The figure shows three views and two pictorial views of one solid part (mm, origin at its lowest corner). Answer the questions. Give positions to 0.01 mm unless a question says otherwise; leave off trailing zeros. Write each loop counter-clockwise with the first axis right and the second up, starting at its lowest first coordinate (ties: lowest second). Pieces come first, ordered by that corner, then holes. Notation, with made-up numbers: (22.5, 69.25) -> (75.5, 69.25) arc R16 cw to (75.5, 94.25) -> close; hole circle Ø4 at (-39.5, 19). An arc over 180 degrees is marked (long way). Answer as CSV lines item,"result". Start each with the question number.
1. The part is cut by section D-D, the plane y = 31. Determine the outline of the cut face in (x, z), and give its area (3 significant figures).
2. The part is cut by section B-B, the plane z = 47.5. Determine the outline of the cut face in (x, y).
3. The part is cut by section A-A, the plane x = 47.5. Determine the outline of the cut face in (y, z), and give its area (3 significant figures).
4. The part is cut by section C-C, the plane y = 9.5. Determine the outline of the cut face in (x, z).
5. For a pull along Z with two mould halves and no side action, classify the marked faces 1, 2, 3 and 4 as pulls with the +Z half, pulls with the -Z half, needs draft (parallel to the pull), parting line crosses it, or undercut.
6. Find the intervals of material crossed by line 1 (X direction, y = 28, z = 47); line 2 (X direction, y = 26, z = 47); line 3 (Y direction, x = 89, z = 58), in increasing order.
7. Given pin 1 (1 mm diameter, centred on x = 24, z = 78.5, fed in from -Y); pin 2 (2 mm diameter, centred on x = 29.5, y = 4.5, fed in from -Z); pin 3 (1.5 mm diameter, centred on y = 13.5, z = 69.5, fed in from +X), each flat-ended and moving along its own axis, determine where each tip first touches the part or whether it passes through.
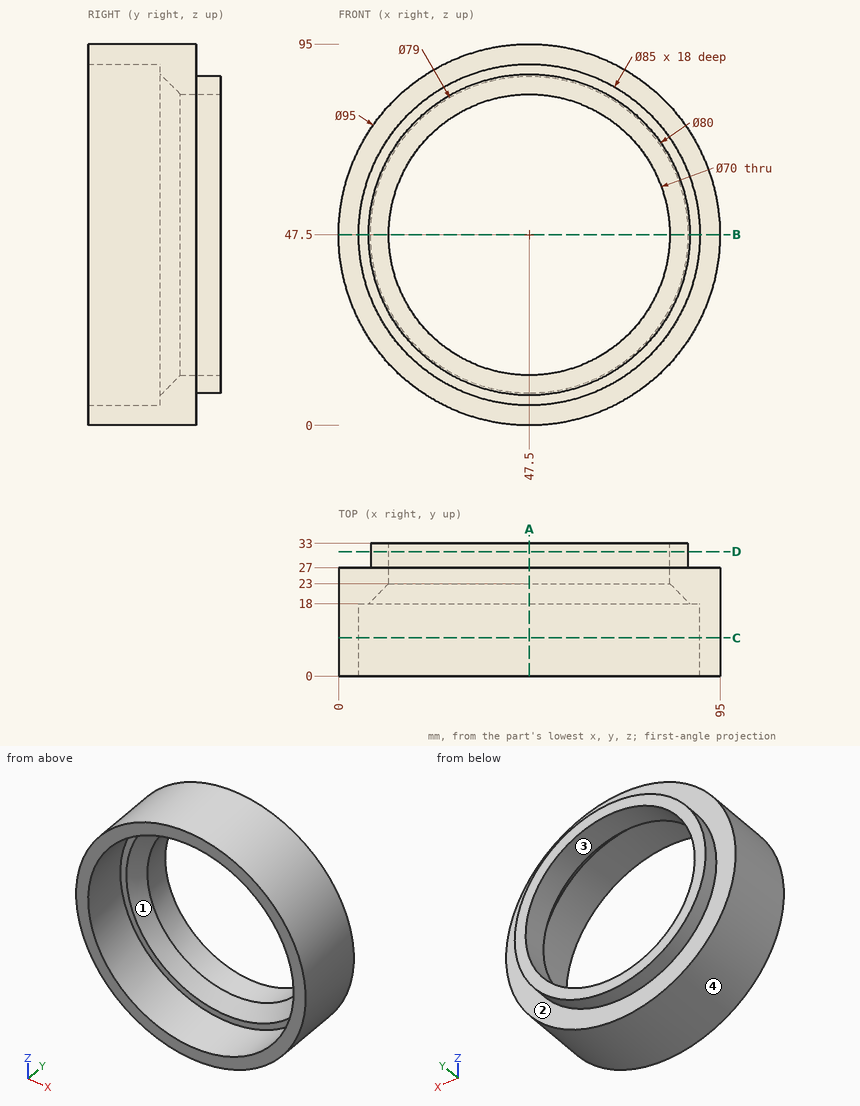
Results found:
1,outline,"circle Ø79 at (47.5, 47.5); hole circle Ø70 at (47.5, 47.5)"
1,area,"1,050 mm²"
2,outline,"(0, 0) -> (5, 0) -> (5, 18) -> (7.5, 18) -> (12.5, 23) -> (12.5, 33) -> (8, 33) -> (8, 27) -> (0, 27) -> close; (82.5, 23) -> (87.5, 18) -> (90, 18) -> (90, 0) -> (95, 0) -> (95, 27) -> (87, 27) -> (87, 33) -> (82.5, 33) -> close"
3,outline,"(0, 0) -> (27, 0) -> (27, 8) -> (33, 8) -> (33, 12.5) -> (23, 12.5) -> (18, 7.5) -> (18, 5) -> (0, 5) -> close; (0, 90) -> (18, 90) -> (18, 87.5) -> (23, 82.5) -> (33, 82.5) -> (33, 87) -> (27, 87) -> (27, 95) -> (0, 95) -> close"
3,area,"434 mm²"
4,outline,"circle Ø95 at (47.5, 47.5); hole circle Ø85 at (47.5, 47.5)"
5,face 1,"undercut"
5,face 2,"needs draft"
5,face 3,"undercut"
5,face 4,"parting line crosses it"
6,line 1,"x = 8 to 12.5, 82.5 to 87"
6,line 2,"x = 0 to 12.5, 82.5 to 95"
6,line 3,"y = 0 to 27"
7,pin 1,"stops at y = 18.6"
7,pin 2,"stops at z = 3.15"
7,pin 3,"stops at x = 89.98"
